Study the drawing (mm; zero at the part's minimum x, y, z) and answer. Coordinates: 2 decimals unless noted, no trailing zeros. Write each loop counter-clockwise with the first axis right and the second up, starting at its lowest first coordinate (ties: lowest second). Pieces come first, ordered by that corner, then holes. Notation, with made-up numbers: (7, 56) -> (49, 56) arc R19 cw to (49, 69) -> close; hole circle Ø6 at (-38.75, -22.5). An arc over 180 degrees is marked (long way). Write item = value, one per line. Start each with the question number.
1) Section C-C (y = 92) is taken. Determine the outline of the cut face in (x, z).
2) Section A-A (z = 130) is taken. Determine the outline of the cut face in (x, y), plus the area to 3 significant figures.
3) Flat-ended cylindrical pins translate along their axes: pin 1 Ø5.5 at (y, z) = (88.5, 68.5) entering from +X; pin 2 Ø4 at (x, z) = (3.5, 34) entering from -Y. Find the tip coordinate at first contact, or state that the pin passes through.
4) Section D-D (z = 25) is taken. Determine the outline of the cut face in (x, y), plus the area to 3 significant figures.
5) Find the intervals of material crossed by line 1 along Y through (x, z) = (7.25, 70); line 2 along Y through (x, z) = (6.5, 130); line 3 along Z through (x, y) = (11.75, 82), in increasing order. Write a range as from..to.
6) Section B-B (x = 5.75) is taken. Determine the outline of the cut face in (y, z).
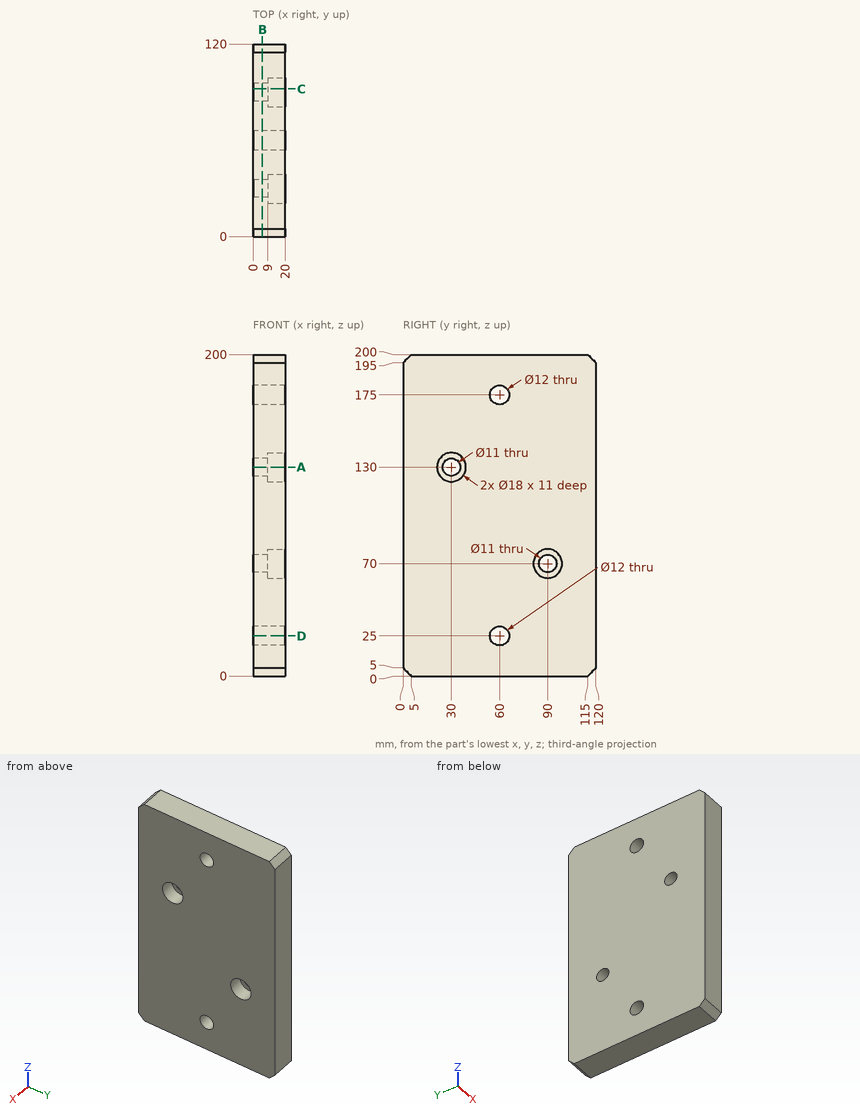
Answer key:
q1.outline = (0, 0) -> (20, 0) -> (20, 61.23) -> (9, 61.23) -> (9, 64.88) -> (0, 64.88) -> close; (0, 75.12) -> (9, 75.12) -> (9, 78.77) -> (20, 78.77) -> (20, 200) -> (0, 200) -> close
q2.outline = (0, 0) -> (20, 0) -> (20, 21) -> (9, 21) -> (9, 24.5) -> (0, 24.5) -> close; (0, 35.5) -> (9, 35.5) -> (9, 39) -> (20, 39) -> (20, 120) -> (0, 120) -> close
q2.area = 2,100 mm^2
q3.pin_1 = through
q3.pin_2 = 0
q4.outline = (0, 0) -> (20, 0) -> (20, 54) -> (0, 54) -> close; (0, 66) -> (20, 66) -> (20, 120) -> (0, 120) -> close
q4.area = 2,160 mm^2
q5.line_1 = 0..84.5, 95.5..120
q5.line_2 = 0..24.5, 35.5..120
q5.line_3 = 0..65.88, 74.12..200
q6.outline = (0, 5) -> (5, 0) -> (115, 0) -> (120, 5) -> (120, 195) -> (115, 200) -> (5, 200) -> (0, 195) -> close; hole circle Ø11 at (30, 130); hole circle Ø12 at (60, 25); hole circle Ø12 at (60, 175); hole circle Ø11 at (90, 70)
